Build history of the part. All positions in model axes, mm. A direction names the side the tool comes from. Give positions to 0.01 mm unless a question says otherwise; leave off trailing zeros. Loops run counter-clockwise (first coordinate to the right, second up) from the corner with the lowest first, then second, coordinate; pieces in that order, holes last. Notation, with made-up numbers: M 76.25,-28 L 90.25,-28 A8 ccw 90.25,-18 Z; hole C 45.5,35.5 d10. An arc over 180 degrees is marked long. Answer in a Markdown table with one row per item. Add a question column.
```python
from build123d import *

# Parameters (mm, degrees)
BASE_PLATE_DEPTH                    = 20
SKETCH1_4_R                         = 15
BEARING_HOUSING_DEPTH               = 10
HOUSING_FILLET_R5_A_R               = 5
HOUSING_FILLET_R5_B_R               = 5
SUPPORT_START                       = 25
SUPPORT_RIB_DEPTH                   = 10
RIB_START                           = 25
RIB_MIRROR_FRONT_PLANE_COPY_1_DEPTH = 10
MOUNTING_HOLE_SKETCH_R              = 5
MOUNTING_HOLE_10_DEPTH              = 89.317608663


with BuildPart() as part:
    # Bracket Profile Sketch → Base Plate (new, symmetric)
    with BuildSketch(Plane.XY):
        Polygon((-50, 0), (0, 0), (0, 10), (-30, 10), (-50, 10), align=None)
        Polygon((0, 10), (0, 0), (50, 0), (50, 10), (30, 10), align=None)
    extrude(amount=BASE_PLATE_DEPTH, both=True)

    # Sketch1_4 → Bearing Housing (add, symmetric)
    # profile 1 of 2: a face of its own
    with BuildSketch(Plane.XY):
        Polygon((-50, 10), (-50, 0), (50, 0), (50, 10), (30, 10), (-30, 10), align=None)
    # profile 2 of 2: a face of its own
    with BuildSketch(Plane.XY):
        with BuildLine():
            Line((-30, 40), (-30, 10))
            Line((-30, 10), (30, 10))
            Line((30, 10), (30, 40))
            ThreePointArc((30, 40), (0, 70), (-30, 40))
        make_face()
        with Locations((0, 40)):
            Circle(SKETCH1_4_R, mode=Mode.SUBTRACT)
    extrude(amount=BEARING_HOUSING_DEPTH, both=True)

    # Housing Fillet R5 A
    housing_fillet_r5_a_edges = [part.edges().sort_by_distance(p)[0] for p in [
        (30, 10, 0),
    ]]
    fillet(housing_fillet_r5_a_edges, radius=HOUSING_FILLET_R5_A_R)

    # Housing Fillet R5 B
    housing_fillet_r5_b_edges = [part.edges().sort_by_distance(p)[0] for p in [
        (-30, 10, 0),
    ]]
    fillet(housing_fillet_r5_b_edges, radius=HOUSING_FILLET_R5_B_R)

    # Support Rib Sketch → Support Rib (add)
    with BuildSketch(Plane(origin=(0, 0, 0), x_dir=(0, 0, -1), z_dir=(1, 0, 0)).offset(SUPPORT_START)):
        Polygon((20, 10), (10, 38), (10, 10), align=None)
    support_rib = extrude(amount=-SUPPORT_RIB_DEPTH)

    # Rib Mirror Right Plane: Support Rib across plane
    add(support_rib.mirror(Plane(origin=(0, 0, 0), x_dir=(0, 0, 1), z_dir=(1, 0, 0))))

    # Rib Mirror Front Plane: Support Rib across plane
    add(support_rib.mirror(Plane.XY))

    # Rib Mirror Front Plane copy 1 sketch → Rib Mirror Front Plane copy 1 (add)
    with BuildSketch(Plane.ZY.offset(RIB_START)):
        Polygon((20, 10), (10, 38), (10, 10), align=None)
    extrude(amount=-RIB_MIRROR_FRONT_PLANE_COPY_1_DEPTH)

    # Mounting Hole Sketch → Mounting Hole _10 (cut, through all)
    with BuildSketch(Plane(origin=(0, 0, 0), x_dir=(1, 0, 0), z_dir=(0, 1, 0))):
        with Locations(Location((-42, 0, 0), (0, 0, 270))):
            Circle(MOUNTING_HOLE_SKETCH_R)
    mounting_hole_10 = extrude(amount=MOUNTING_HOLE_10_DEPTH, mode=Mode.SUBTRACT)

    # Mounting Hole Mirror: Mounting Hole _10 across plane
    add(mounting_hole_10.mirror(Plane(origin=(0, 0, 0), x_dir=(0, 0, 1), z_dir=(1, 0, 0))), mode=Mode.SUBTRACT)


solid = part.part
```
(1) Wall check: line 1 (Z direction, x = -42, y = 5); line 2 (X direction, y = 3.5, z = 0); line 3 (X direction, y = 8.5, z = 2). Give the ranges that are in metal, low to high.
(2) Slice it at D-D, the plane x = 0. Give the cut face in (y, z).
(3) Tool access for faces 4 (the flat face through (-40, 10, 5)), 5 (the flat face through (0, 10, -15)), 6 (the flat face through (15, 18, 13)): list every direction of +Z, -Z, +X, -X, +Y, -Y with a clear straight run to the whole face (end or side of a thin tool).
(4) Slice it at B-B, the plane z = -7. Give the cut face in (x, y), then the cut area to 3 significant figures.
(5) Slice it at C-C, the plane z = 2.5. Give the cut face in (x, y), then the cut area to 3 significant figures.
(6) Pull direction X, two halves, no side cores. Call faces 1 (the flat face through (25, 18, 13)), 2 (the flat face through (-11, 29, 10)), 3 (the flat face through (20, 24, -15)): +X half, -X half, draft (parallel to the pull), parting line (faces both ways), or undercut.
(7) Pin check, flat tips, straight feed: pin 1 (6 mm diameter, centred on y = 26.5, z = -8.5, fed in from +X); pin 2 (11 mm diameter, centred on y = 25, z = -12.5, fed in from -X); pin 3 (11.5 mm diameter, centred on x = -42, z = 0, fed in from +Y). Stop position of each tip, or through.
(8) Slice it at A-A, the plane x = 42. Give the cut face in (y, z), then the cut area to 3 significant figures.
Solution:
| question | item | result |
|---|---|---|
| 1 | line 1 | -20 to -5, 5 to 20 |
| 1 | line 2 | -50 to -47, -37 to 37, 47 to 50 |
| 1 | line 3 | -50 to -46.58, -37.42 to 37.42, 46.58 to 50 |
| 2 | outline | M 0,-20 L 10,-20 L 10,-10 L 25,-10 L 25,10 L 10,10 L 10,20 L 0,20 Z; M 55,-10 L 70,-10 L 70,10 L 55,10 Z |
| 3 | face 4 | -X, +Y |
| 3 | face 5 | -Z, +Y |
| 3 | face 6 | +Z, +Y |
| 4 | outline | M -50,0 L 50,0 L 50,10 L 35,10 A5 cw 30,15 L 30,40 A30 ccw -30,40 L -30,15 A5 cw -35,10 L -50,10 Z; hole C 0,40 d30 |
| 4 | area | 3,520 mm^2 |
| 5 | outline | M -50,0 L -46.33,0 L -46.33,10 L -50,10 Z; M -37.67,0 L 37.67,0 L 37.67,10 L 35,10 A5 cw 30,15 L 30,40 A30 ccw -30,40 L -30,15 A5 cw -35,10 L -37.67,10 Z; M 46.33,0 L 50,0 L 50,10 L 46.33,10 Z; hole C 0,40 d30 |
| 5 | area | 3,340 mm^2 |
| 6 | face 1 | +X half |
| 6 | face 2 | undercut |
| 6 | face 3 | draft |
| 7 | pin 1 | x = 30 |
| 7 | pin 2 | x = -30 |
| 7 | pin 3 | y = 10 |
| 8 | outline | M 0,-20 L 10,-20 L 10,-5 L 0,-5 Z; M 0,5 L 10,5 L 10,20 L 0,20 Z |
| 8 | area | 300 mm^2 |
